The model under review builds one solid part; all positions refer to its coordinate system, in mm. A direction names the side the tool comes from. Give positions to 0.01 mm unless a question says otherwise; leave off trailing zeros. Order: outer loops, then holes, each group sorted by start corner. A loop starts at its lowest first (then second) coordinate and runs counter-clockwise, first axis right, second up.
```python
from build123d import *

# Parameters (mm, degrees)
SKETCH_1_R          = 7
EXTRUDE_1_DEPTH     = 30
SKETCH_2_R          = 25
EXTRUDE_2_DEPTH     = 3
SKETCH_3_W          = 60
SKETCH_3_H          = 60
EXTRUDE_3_DEPTH     = 8
SKETCH_4_R          = 30
EXTRUDE_4_DEPTH     = 41
SKETCH_5_W          = 60
SKETCH_5_H          = 60
EXTRUDE_5_DEPTH     = 31
SKETCH_6_W          = 7.340334956
SKETCH_6_H          = 80
CUT_EXTRUDE_1_REACH = 92.554
SKETCH_7_R          = 2.75
CUT_EXTRUDE_START   = -5
SKETCH_8_R          = 25
CUT_EXTRUDE_2_DEPTH = 5
CUT_EXTRUDE_START_2 = -25
SKETCH_9_R          = 7
CUT_EXTRUDE_3_DEPTH = 25


with BuildPart() as part:
    # 草图1 → 凸台-拉伸1 (new body)
    with BuildSketch(Plane.XY):
        Circle(SKETCH_1_R)
    extrude(amount=EXTRUDE_1_DEPTH)

    # 草图2 → 凸台-拉伸2 (add)
    with BuildSketch(Plane.XY.offset(30)):
        Circle(SKETCH_2_R)
    extrude(amount=EXTRUDE_2_DEPTH)

    # 草图3 → 凸台-拉伸3 (add)
    with BuildSketch(Plane.XY.offset(33)):
        Rectangle(SKETCH_3_W, SKETCH_3_H)
    extrude(amount=EXTRUDE_3_DEPTH)

    # 草图4 → 凸台-拉伸4 (add)
    with BuildSketch(Plane.XY.offset(41)):
        Circle(SKETCH_4_R)
    extrude(amount=EXTRUDE_4_DEPTH)

    # 草图5 → 凸台-拉伸5 (add)
    with BuildSketch(Plane.XY.offset(82)):
        Rectangle(SKETCH_5_W, SKETCH_5_H)
    extrude(amount=EXTRUDE_5_DEPTH)

    # 草图6 → 切除-旋转1 (revolve, cut)
    with BuildSketch(Plane(origin=(0, 0, 0), x_dir=(1, 0, 0), z_dir=(0, 1, 0))):
        with Locations((-43.670167478, -73)):
            Rectangle(SKETCH_6_W, SKETCH_6_H)
    revolve(axis=Axis((0, 0, 82), (0, 0, -1)), mode=Mode.SUBTRACT)

    # 草图7 → 切除-拉伸1 (cut, up to next)
    with BuildSketch(Plane(origin=(0, 0, 33), x_dir=(-1, 0, 0), z_dir=(0, 0, -1)), mode=Mode.PRIVATE) as cut_extrude_1_sk1:
        with Locations((-24.748737342, 24.748737342)):
            Circle(SKETCH_7_R)
    cut_extrude_1_tool1 = extrude(cut_extrude_1_sk1.sketch, amount=-CUT_EXTRUDE_1_REACH, mode=Mode.PRIVATE) & part.part
    # 草图7 → 切除-拉伸1 (cut, up to next)
    with BuildSketch(Plane(origin=(0, 0, 33), x_dir=(-1, 0, 0), z_dir=(0, 0, -1)), mode=Mode.PRIVATE) as cut_extrude_1_sk2:
        with Locations(Location((24.748737342, 24.748737342, 0), (0, 0, 180))):
            Circle(SKETCH_7_R)
    cut_extrude_1_tool2 = extrude(cut_extrude_1_sk2.sketch, amount=-CUT_EXTRUDE_1_REACH, mode=Mode.PRIVATE) & part.part
    # 草图7 → 切除-拉伸1 (cut, up to next)
    with BuildSketch(Plane(origin=(0, 0, 33), x_dir=(-1, 0, 0), z_dir=(0, 0, -1)), mode=Mode.PRIVATE) as cut_extrude_1_sk3:
        with Locations(Location((-24.748737342, -24.748737342, 0), (0, 0, 180))):
            Circle(SKETCH_7_R)
    cut_extrude_1_tool3 = extrude(cut_extrude_1_sk3.sketch, amount=-CUT_EXTRUDE_1_REACH, mode=Mode.PRIVATE) & part.part
    # 草图7 → 切除-拉伸1 (cut, up to next)
    with BuildSketch(Plane(origin=(0, 0, 33), x_dir=(-1, 0, 0), z_dir=(0, 0, -1)), mode=Mode.PRIVATE) as cut_extrude_1_sk4:
        with Locations((24.748737342, -24.748737342)):
            Circle(SKETCH_7_R)
    cut_extrude_1_tool4 = extrude(cut_extrude_1_sk4.sketch, amount=-CUT_EXTRUDE_1_REACH, mode=Mode.PRIVATE) & part.part
    add(cut_extrude_1_tool1.solids().sort_by_distance((24.748737, 24.748737, 33))[0], mode=Mode.SUBTRACT)
    add(cut_extrude_1_tool2.solids().sort_by_distance((-24.748737, 24.748737, 33))[0], mode=Mode.SUBTRACT)
    add(cut_extrude_1_tool3.solids().sort_by_distance((24.748737, -24.748737, 33))[0], mode=Mode.SUBTRACT)
    add(cut_extrude_1_tool4.solids().sort_by_distance((-24.748737, -24.748737, 33))[0], mode=Mode.SUBTRACT)

    # 草图8 → 切除-拉伸2 (cut)
    with BuildSketch(Plane.XY.offset(113).offset(CUT_EXTRUDE_START)):
        Circle(SKETCH_8_R)
    extrude(amount=CUT_EXTRUDE_2_DEPTH, mode=Mode.SUBTRACT)

    # 草图9 → 切除-拉伸3 (cut)
    with BuildSketch(Plane.XY.offset(108).offset(CUT_EXTRUDE_START_2)):
        Circle(SKETCH_9_R)
    extrude(amount=CUT_EXTRUDE_3_DEPTH, mode=Mode.SUBTRACT)


solid = part.part
```
Item 1: Clearance check with flat-ended pins moving along their axes: pin 1 Ø4.5 at (x, y) = (-24.75, 24.75) entering from -Z; pin 2 Ø8.5 at (x, y) = (0, 0) entering from +Z; pin 3 Ø8 at (x, z) = (6, 71.5) entering from -Y. State where each tip first meets the part, or that it passes through.
Values found:
pin 1: stops at z = 82
pin 2: stops at z = 83
pin 3: stops at y = -29.93
Item 2: Draft analysis for pull direction X (two halves, no side actions). For faces 4 (the cylindrical face through (26, -22.3, 36.9)), 5 (the cylindrical face through (28.31, -28.26, 36.94)), 6 (the flat face through (-30, 0, 37)), state which applies: released by +X, released by -X, zero draft, split by the parting line, or undercut.
Values found:
face 4: undercut
face 5: released by +X
face 6: released by -X
Item 3: Take a section at A-A (z = 103.5). Give the boundary of the cut face in (x, y), and give its area (3 significant figures).
Values found:
outline: (-30, -26.46) arc R40 ccw to (-26.46, -30) - (26.46, -30) arc R40 ccw to (30, -26.46) - (30, 26.46) arc R40 ccw to (26.46, 30) - (-26.46, 30) arc R40 ccw to (-30, 26.46) - close; hole circle Ø14 at (0, 0)
area: 3,420 mm2
Item 4: For line 1 (Z direction, x = 19.5, y = 24); line 2 (Y direction, x = 0, z = 98.25); line 3 (Z direction, x = 5, y = 11.5), list the stretches that pass through material, from the lowest coordinate up.
Values found:
line 1: z = 33 to 41, 82 to 113
line 2: y = -30 to -7, 7 to 30
line 3: z = 30 to 108
Item 5: Take a section at C-C (y = 13). Give the boundary of the cut face in (x, z), and give its area (3 significant figures).
Values found:
outline: (-30, 33) - (-21.35, 33) - (-21.35, 30) - (21.35, 30) - (21.35, 33) - (30, 33) - (30, 41) - (27.04, 41) - (27.04, 82) - (30, 82) - (30, 113) - (21.35, 113) - (21.35, 108) - (-21.35, 108) - (-21.35, 113) - (-30, 113) - (-30, 82) - (-27.04, 82) - (-27.04, 41) - (-30, 41) - close
area: 4,470 mm2
Item 6: For faces 1 (the cylindrical face through (-27.37, -23.92, 36.94)), 2 (the flat face through (-23, 24, 82)), 3 (the flat face through (0, 0, 83)), list the 3-axis set-ups (+Z, -Z, +X, -X, +Y, -Y) from which the entire face can be reached by the end or side of a thin tool; tool diameter is ignored.
Values found:
face 1: -Z
face 2: -X, +Y
face 3: +Z
Item 7: Take a section at B-B (x = 10). Give the boundary of the cut face in (y, z), and give its area (3 significant figures).
Values found:
outline: (-30, 33) - (-22.91, 33) - (-22.91, 30) - (22.91, 30) - (22.91, 33) - (30, 33) - (30, 41) - (28.28, 41) - (28.28, 82) - (30, 82) - (30, 113) - (22.91, 113) - (22.91, 108) - (-22.91, 108) - (-22.91, 113) - (-30, 113) - (-30, 82) - (-28.28, 82) - (-28.28, 41) - (-30, 41) - close
area: 4,570 mm2
Item 8: Take a section at D-D (z = 80.5). Give the boundary of the cut face in (x, y), and give its area (3 significant figures).
Values found:
outline: circle Ø60 at (0, 0)
area: 2,830 mm2
